Geometry check sheet. Reference: the model listing, model coordinates, mm. Face numbers are marked on the shaded views. A direction names the side the tool comes from. Give positions to 0.01 mm unless a question says otherwise; leave off trailing zeros. Order: outer loops, then holes, each group sorted by start corner. A loop starts at its lowest first (then second) coordinate and runs counter-clockwise, first axis right, second up. Notation, with made-up numbers: (-6.75, 9) - (22.25, 9) arc R14 ccw to (22.25, 20) - close; hole circle Ø1 at (72, -37). An arc over 180 degrees is marked (long way). Put each result on its own line as item: value. Start each with the question number.
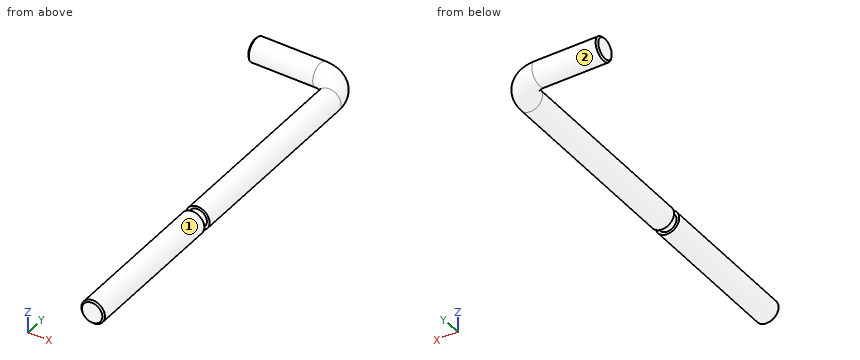
```python
from build123d import *

# Parameters (mm, degrees)
SKETCH2_R     = 2.25
SKETCH3_W     = 0.5
SKETCH3_H     = 1.5
CHAMFER1_SIZE = 0.3


with BuildPart() as part:
    # Sweep1: sweep along a path in Sketch1
    with BuildLine(Plane.XY) as sweep1_path:
        Line((0, 0), (0, 68.5))
        ThreePointArc((0, 68.5), (-1.464466094, 72.035533906), (-5, 73.5))
        Line((-5, 73.5), (-17.5, 73.5))
    # Sketch2 → Sweep1 (sweep)
    with BuildSketch(Plane(origin=(0, 0, 0), x_dir=(1, 0, 0), z_dir=(0, 1, 0))):
        Circle(SKETCH2_R)
    sweep(path=sweep1_path.line)

    # Sketch3 → Cut-Revolve1 (revolve, cut)
    with BuildSketch(Plane(origin=(0, 0, 0), x_dir=(0, 0, -1), z_dir=(1, 0, 0))):
        with Locations((2, 29.75)):
            Rectangle(SKETCH3_W, SKETCH3_H)
    revolve(axis=Axis((0, 0, 0), (0, 1, 0)), mode=Mode.SUBTRACT)

    # Chamfer1
    chamfer1_edges = [part.edges().sort_by_distance(p)[0] for p in [
        (-2.25, 0, 0),
        (-17.5, 71.25, 0),
    ]]
    chamfer(chamfer1_edges, length=CHAMFER1_SIZE)


solid = part.part
```
Item 1: Thickness scan on line 1 along X through (y, z) = (64.5, 1.15); line 2 along Y through (x, z) = (-0.5, 1.8); line 3 along Y through (x, z) = (-14, 0). Record the ranges inside material, lowest first.
Item 2: Cross-section at A-A (z = 0). Enter the section's corners in (x, y).
Item 3: Cross-section at C-C (x = -7.5). Enter the section's corners in (y, z).
Item 4: Set-up check for the marked faces 1 and 2: record each of +Z, -Z, +X, -X, +Y, -Y from which the full face is reachable in a straight line by a thin tool's end or side.
Item 5: Cross-section at B-B (y = 14.5). Enter the section's corners in (x, z), and give its area (3 significant figures).
Item 6: Gauge pin test, flat ends, axial feed: pin 1 Ø4 at (x, y) = (-4, 16.5) entering from +Z; pin 2 Ø1.5 at (y, z) = (18.5, 0.5) entering from -X. Record the tip position at first contact, or that the pin passes through.
Recorded:
1. line 1: x = -1.93 to 1.93
1. line 2: y = 0 to 29, 30.5 to 72.98
1. line 3: y = 71.25 to 75.75
2. outline: (-17.5, 71.55) - (-17.2, 71.25) - (-5, 71.25) arc R2.75 cw to (-2.25, 68.5) - (-2.25, 30.5) - (-1.75, 30.5) - (-1.75, 29) - (-2.25, 29) - (-2.25, 0.3) - (-1.95, 0) - (1.95, 0) - (2.25, 0.3) - (2.25, 29) - (1.75, 29) - (1.75, 30.5) - (2.25, 30.5) - (2.25, 68.5) arc R7.25 ccw to (-5, 75.75) - (-17.2, 75.75) - (-17.5, 75.45) - close
3. outline: circle Ø4.5 at (73.5, 0)
4. face 1: -Y
4. face 2: -X
5. outline: circle Ø4.5 at (0, 0)
5. area: 15.9 mm^2
6. pin 1: stops at z = 1.03
6. pin 2: stops at x = -2.25
